Design review of the part built by this model. Coordinates are the model's own, in mm. A direction names the side the tool comes from. Give positions to 0.01 mm unless a question says otherwise; leave off trailing zeros. Write each loop counter-clockwise with the first axis right and the second up, starting at its lowest first coordinate (ties: lowest second). Pieces come first, ordered by that corner, then holes. Notation, with made-up numbers: (13, -4.5) -> (34, -4.5) arc R31 ccw to (34, 23.5) -> close; hole circle Ø5 at (89, 57). An arc over 180 degrees is marked (long way). Write each question's results on one line, items separated by ' | '. Start each with the question number.
(1) Clearance check with flat-ended pins moving along their axes: pin 1 (4.5 mm diameter, centred on x = -5.08, y = 1.25, fed in from +Z); pin 2 (2 mm diameter, centred on y = -1, z = 8.5, fed in from +X); pin 3 (3.5 mm diameter, centred on x = 0, z = 6.25, fed in from +Y). State where each tip first meets the part, or that it passes through.
(2) Take a section at D-D (y = -3.5). State the section outline as (x, z) points, plus the area to 3 significant figures.
(3) Take a section at C-C (z = 6.25). State the section outline as (x, y) points.
(4) Take a section at B-B (y = 1.25). State the section outline as (x, z) points.
(5) Take a section at A-A (x = 0). State the section outline as (y, z) points.
(6) To check wall thickness, follow probe 1 along Y at (x, z) = (2.5, 6); probe 2 along X at (y, z) = (-3.3, 6.25); probe 3 along Z at (x, y) = (1, 0.5). State the ranges of each line that lie inside material, in increasing order.
(7) Mouldability with a two-part tool opening along Y and no side actions: class faces 3 (the face through (0.178, -3.764, 9.532)), 4 (the face through (0, -4.75, 4)), 5 (the face through (-6.828, 1.327, 1.232)) as released by +Y, released by -Y, zero draft, split by the parting line, or undercut.
(8) For faces 1 (the face through (0, 1, 2.5)), 2 (the face through (0.07, -3.76, 7.75)), list the 3-axis set-ups (+Z, -Z, +X, -X, +Y, -Y) from which the entire face can be reached by the end or side of a thin tool; tool diameter is ignored.
from build123d import *

# Parameters (mm, degrees)
SKETCH_1_R      = 1.75
EXTRUDE_1_DEPTH = 2.5
SKETCH_2_R      = 1.5
EXTRUDE_2_DEPTH = 2
FILLET_1_R      = 2


with BuildPart() as part:
    # 草图1 → 凸台-拉伸1 (new body)
    with BuildSketch(Plane.XY):
        with BuildLine():
            Line((-9.55, -4.75), (9.55, -4.75))
            Line((9.55, -4.75), (9.55, 1.75))
            ThreePointArc((9.55, 1.75), (8.671320344, 3.871320344), (6.55, 4.75))
            Line((6.55, 4.75), (-6.55, 4.75))
            ThreePointArc((-6.55, 4.75), (-8.671320344, 3.871320344), (-9.55, 1.75))
            Line((-9.55, 1.75), (-9.55, -4.75))
        make_face()
        with Locations((4.920618816, 1.25)):
            Circle(SKETCH_1_R, mode=Mode.SUBTRACT)
        with Locations((-5.079381184, 1.25)):
            Circle(SKETCH_1_R, mode=Mode.SUBTRACT)
    extrude(amount=EXTRUDE_1_DEPTH)

    # 草图2 → 凸台-拉伸2 (add)
    with BuildSketch(Plane.XZ.offset(4.75)):
        with BuildLine():
            Line((-9.55, 2.5), (9.55, 2.5))
            ThreePointArc((9.55, 2.5), (0, 9.53394201), (-9.55, 2.5))
        make_face()
        with Locations(Location((0, 6.25, 0), (0, 0, 270))):
            Circle(SKETCH_2_R, mode=Mode.SUBTRACT)
    extrude(amount=-EXTRUDE_2_DEPTH)

    # 圆角1
    fillet_1_edges = [part.edges().sort_by_distance(p)[0] for p in [
        (0, -4.75, 0),
    ]]
    fillet(fillet_1_edges, radius=FILLET_1_R)


solid = part.part
Report:
1) pin 1: z = 2.5 | pin 2: through | pin 3: y = -2.75
2) outline: (-9.55, 0.15) -> (9.55, 0.15) -> (9.55, 2.5) arc R10 ccw to (-9.55, 2.5) -> close; hole circle Ø3 at (0, 6.25) | area: 137 mm2
3) outline: (-7.41, -4.75) -> (-1.5, -4.75) -> (-1.5, -2.75) -> (-7.41, -2.75) -> close; (1.5, -4.75) -> (7.41, -4.75) -> (7.41, -2.75) -> (1.5, -2.75) -> close
4) outline: (-9.55, 0) -> (-6.83, 0) -> (-6.83, 2.5) -> (-9.55, 2.5) -> close; (-3.33, 0) -> (3.17, 0) -> (3.17, 2.5) -> (-3.33, 2.5) -> close; (6.67, 0) -> (9.55, 0) -> (9.55, 2.5) -> (6.67, 2.5) -> close
5) outline: (-4.75, 2) arc R2 ccw to (-2.75, 0) -> (4.75, 0) -> (4.75, 2.5) -> (-2.75, 2.5) -> (-2.75, 4.75) -> (-4.75, 4.75) -> close; (-4.75, 7.75) -> (-2.75, 7.75) -> (-2.75, 9.53) -> (-4.75, 9.53) -> close
6) probe 1: -4.75 to -2.75 | probe 2: -7.41 to -1.5, 1.5 to 7.41 | probe 3: 0 to 2.5
7) face 3: zero draft | face 4: released by -Y | face 5: undercut
8) face 1: +Z, +X, -X, +Y | face 2: +Y, -Y
